```python
from build123d import *

# Parameters (mm, degrees)
SKETCH1_R           = 3.175
BOSS_EXTRUDE1_DEPTH = 3.175


with BuildPart() as part:
    # Sketch1 → Boss-Extrude1 (new body)
    with BuildSketch(Plane(origin=(0, 0, 0), x_dir=(1, 0, 0), z_dir=(0, 1, 0))):
        with BuildLine():
            Line((0, 7.9502), (34.925, 7.9502))
            ThreePointArc((34.925, 7.9502), (42.8752, 0), (34.925, -7.9502))
            Line((34.925, -7.9502), (15.497902875, -7.9502))
            ThreePointArc((15.497902875, -7.9502), (10.963581061, -9.854705012), (9.149145427, -14.425813956))
            Line((9.149145427, -14.425813956), (12.7, -57.15))
            ThreePointArc((12.7, -57.15), (0, -69.85), (-12.7, -57.15))
            Line((-12.7, -57.15), (-7.9502, 0))
            ThreePointArc((-7.9502, 0), (-5.621640332, 5.621640332), (0, 7.9502))
        make_face()
        with Locations(Location((34.925, 0, 0), (0, 0, 270))):
            Circle(SKETCH1_R, mode=Mode.SUBTRACT)
        with Locations(Location((0, 0, 0), (0, 0, 270))):
            Circle(SKETCH1_R, mode=Mode.SUBTRACT)
        with Locations(Location((0, -57.15, 0), (0, 0, 270))):
            Circle(SKETCH1_R, mode=Mode.SUBTRACT)
    extrude(amount=BOSS_EXTRUDE1_DEPTH)


solid = part.part
```
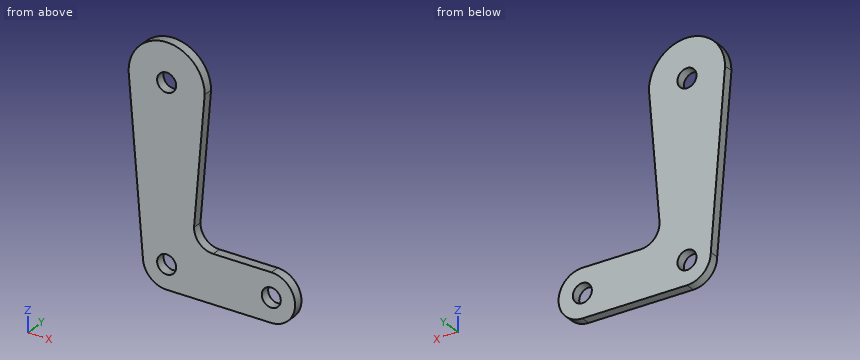
Check sheet for the modelled part. Datum: model origin and axes. Units: mm. Give positions to 0.01 mm unless a question says otherwise; leave off trailing zeros. Order: outer loops, then holes, each group sorted by start corner. A loop starts at its lowest first (then second) coordinate and runs counter-clockwise, first axis right, second up. Notation, with made-up numbers: M 75,-22.75 L 116,-22.75 A22 cw 116,-4.75 Z; hole C -23.75,32 d10. An arc over 180 degrees is marked long. Answer in a Markdown table with one row per item. Add a question column.
Q1. Gauge pin test, flat ends, axial feed: pin 1 Ø1.5 at (y, z) = (2, 61.5) entering from +X; pin 2 Ø1 at (x, y) = (11.5, 1) entering from +Z; pin 3 Ø1.6 at (x, y) = (30, 1.5) entering from +Z; pin 4 Ø5 at (x, z) = (30, 1) entering from -Y. Record the tip position at first contact, or that the pin passes through.
Q2. Thickness scan on L1, parallel to X at y = 2.1, z = 57.15 (3 decimals); L2, parallel to X at y = 2.65, z = -2; L3, parallel to X at y = 0.95, z = 0 (3 decimals). Record the ranges inside material, lowest first.
Q3. Sectioned sample at C-C, the plane z = 11. Record the boundary of the cut face in (x, y) (3 decimals), and give its area (3 significant figures).
Q4. Sectioned sample at B-B, the plane x = 30.5. Record the boundary of the cut face in (y, z) (3 decimals).
Q5. Sectioned sample at A-A, the plane y = 2. Record the boundary of the cut face in (x, z) (3 decimals).
Verdict:
| question | item | result |
|---|---|---|
| 1 | pin 1 | x = 12.18 |
| 1 | pin 2 | z = 63.5 |
| 1 | pin 3 | z = 7.95 |
| 1 | pin 4 | y = 0 |
| 2 | L1 | -12.7 to -3.175, 3.175 to 12.7 |
| 2 | L2 | -7.69 to -2.47, 2.47 to 32.46, 37.39 to 42.62 |
| 2 | L3 | -7.95 to -3.175, 3.175 to 31.75, 38.1 to 42.875 |
| 3 | outline | M -8.864,0 L 10.073,0 L 10.073,3.175 L -8.864,3.175 Z |
| 3 | area | 60.1 mm² |
| 4 | outline | M 0,-7.95 L 3.175,-7.95 L 3.175,7.95 L 0,7.95 Z |
| 5 | outline | M -12.7,57.15 L -7.95,0 A7.95 ccw 0,-7.95 L 34.925,-7.95 A7.95 ccw 34.925,7.95 L 15.498,7.95 A6.35 cw 9.149,14.426 L 12.7,57.15 A12.7 ccw Z; hole C 0,0 d6.35; hole C 0,57.15 d6.35; hole C 34.925,0 d6.35 |
